```python
from build123d import *

# Parameters (mm, degrees)
SKETCH1_R           = 2.5
BOSS_EXTRUDE1_DEPTH = 20
SKETCH2_R           = 3.75
BOSS_EXTRUDE2_DEPTH = 2
SKETCH3_R           = 2.25
BOSS_EXTRUDE3_DEPTH = 30
SKETCH7_R           = 4
SKETCH7_R_2         = 2
CUT_EXTRUDE1_DEPTH  = 33.436476381


with BuildPart() as part:
    # Sketch1 → Boss-Extrude1 (new body)
    with BuildSketch(Plane(origin=(0, 0, 0), x_dir=(1, 0, 0), z_dir=(0, 1, 0))):
        with Locations(Location((0, 0, 0), (0, 0, 270))):
            Circle(SKETCH1_R)
    extrude(amount=BOSS_EXTRUDE1_DEPTH)

    # Sketch2 → Boss-Extrude2 (add)
    with BuildSketch(Plane.XZ):
        with Locations(Location((0, 0, 0), (0, 0, 270))):
            Circle(SKETCH2_R)
    extrude(amount=BOSS_EXTRUDE2_DEPTH)

    # Sketch3 → Boss-Extrude3 (add)
    with BuildSketch(Plane.XZ.offset(2)):
        with Locations(Location((0, 0, 0), (0, 0, 270))):
            Circle(SKETCH3_R)
    extrude(amount=BOSS_EXTRUDE3_DEPTH)

    # Sketch4 → Revolve1 (revolve)
    with BuildSketch(Plane.XY, mode=Mode.PRIVATE) as revolve1_sk:
        with BuildLine():
            Line((1, 20), (0, 20))
            Line((0, 20), (0, 21))
            ThreePointArc((0, 21), (0.707106781, 20.707106781), (1, 20))
        make_face()
    revolve(revolve1_sk.sketch.rotate(Axis((0, 20, 0), (0, 1, 0)), 90), axis=Axis((0, 20, 0), (0, 1, 0)))

    # Sketch5 → Cut-Revolve1 (revolve, cut)
    with BuildSketch(Plane(origin=(0, 0, 0), x_dir=(0, 0, -1), z_dir=(1, 0, 0)), mode=Mode.PRIVATE) as cut_revolve1_sk:
        Polygon((1.0823922, 20), (2.5, 16.577592024), (2.5, 20), align=None)
    revolve(cut_revolve1_sk.sketch.rotate(Axis((0, 15, 0), (0, -1, 0)), 90), axis=Axis((0, 15, 0), (0, -1, 0)), mode=Mode.SUBTRACT)

    # Sketch6 → Revolve2 (revolve)
    with BuildSketch(Plane(origin=(0, 0, 0), x_dir=(0, 0, -1), z_dir=(1, 0, 0))):
        with BuildLine():
            Line((1.0823922, 20), (0.923879533, 20.382683432))
            ThreePointArc((0.923879533, 20.382683432), (0.98078528, 20.195090322), (1, 20))
            Line((1, 20), (1.0823922, 20))
        make_face()
    revolve(axis=Axis((0, 16, 0), (0, 1, 0)))

    # Sketch7 → Cut-Extrude1 (cut, through all)
    with BuildSketch(Plane(origin=(0, 0, 0), x_dir=(1, 0, 0), z_dir=(0, 1, 0))):
        Circle(SKETCH7_R)
        with Locations(Location((0, 0, 0), (0, 0, 90))):
            Circle(SKETCH7_R_2, mode=Mode.SUBTRACT)
    extrude(amount=CUT_EXTRUDE1_DEPTH, mode=Mode.SUBTRACT)


solid = part.part
```
For this review, take the finished solid that the model builds, in its own axes (mm). A direction names the side the tool comes from. Round coordinates to 2 decimals unless told otherwise and drop trailing zeros. Write each loop counter-clockwise with the first axis right and the second up, starting at its lowest first coordinate (ties: lowest second). Pieces come first, ordered by that corner, then holes. Notation, with made-up numbers: (-2, 74) - (34, 74) arc R21 cw to (34, 87) - close; hole circle Ø11 at (37.25, 46.25). An arc over 180 degrees is marked (long way). Write each question's results on one line, items separated by ' | '.
Item 1: Take a section at D-D on y = -10.5. State the section outline as (x, z) points.
Calculated:
outline: circle Ø4.5 at (0, 0)
Item 2: Take a section at C-C on x = 3.25. State the section outline as (y, z) points.
Calculated:
outline: (-2, -1.87) - (0, -1.87) - (0, 1.87) - (-2, 1.87) - close
Item 3: To check wall thickness, follow line 1 along Y through (x, z) = (0.25, -3); line 2 along Z through (x, y) = (-0.5, -14.5); line 3 along X through (y, z) = (-26, 0). State the ranges of each line that lie inside material, in increasing order. Write a range as from..to.
Calculated:
line 1: y = -2..0 | line 2: z = -2.19..2.19 | line 3: x = -2.25..2.25
Item 4: For pin 1 (2 mm diameter, centred on x = 1, z = 1, fed in from +Y); pin 2 (1 mm diameter, centred on x = 2.5, y = -11.5, fed in from +Z); pin 3 (1 mm diameter, centred on x = 1.5, y = 7, fed in from -Z), all flat-tipped, find the tip position at first contact; note any pin that passes through.
Calculated:
pin 1: stops at y = 20.91 | pin 2: stops at z = 1.03 | pin 3: stops at z = -1.73
Item 5: For faces 1 (the face through (0, -32, 0)), 2 (the face through (2, 0, 2)), 3 (the face through (0.676, -16.79, -2.146)), list the 3-axis set-ups (+Z, -Z, +X, -X, +Y, -Y) from which the entire face can be reached by the end or side of a thin tool; tool diameter is ignored.
Calculated:
face 1: +Z, -Z, +X, -X, -Y | face 2: +Y | face 3: -Y
Item 6: Take a section at B-B on z = 3. State the section outline as (x, y) points.
Calculated:
outline: (-2.25, -2) - (2.25, -2) - (2.25, 0) - (-2.25, 0) - close
Item 7: Take a section at A-A on y = 7. State the section outline as (x, z) points, then the cut area to 3 significant figures.
Calculated:
outline: circle Ø4 at (0, 0) | area: 12.6 mm^2
